The model under review builds one solid part; all positions refer to its coordinate system, in mm. A direction names the side the tool comes from. Round coordinates to 2 decimals unless told otherwise and drop trailing zeros. Order: outer loops, then holes, each group sorted by start corner. A loop starts at its lowest first (then second) coordinate and runs counter-clockwise, first axis right, second up. Notation, with made-up numbers: M 79,29.5 L 96,29.5 A26 cw 96,54.5 Z; hole C 25.25,73.5 d3. An arc over 180 degrees is marked long. Answer as CSV lines item,"result". Start each with the question number.
from build123d import *

# Parameters (mm, degrees)
SKETCH_1_W                  = 58
SKETCH_1_H                  = 103.5
EXTRUDE_1_DEPTH             = 12
HOLE_WIZARD_M4_1_D          = 3.3
SKETCH_5_R                  = 20
CUT_EXTRUDE_1_DEPTH         = 61.523239338
SKETCH_6_W                  = 58
SKETCH_6_H                  = 58
EXTRUDE_2_DEPTH             = 10
SKETCH_10_W                 = 48
SKETCH_10_H                 = 10
CUT_EXTRUDE_2_DEPTH         = 146
CHAMFER_1_SIZE              = 3
CUT_EXTRUDE_5_DEPTH         = 86.56320763
CUT_EXTRUDE_5_DEPTH_BACK    = 86.56320763
SKETCH_15_W                 = 130
SKETCH_15_H                 = 14
EXTRUDE_3_DEPTH             = 12
SKETCH_16_W                 = 40
SKETCH_16_H                 = 14
EXTRUDE_4_DEPTH             = 60
EXTRUDE_START               = -40
SKETCH_17_W                 = 12
SKETCH_17_H                 = 100
EXTRUDE_5_DEPTH             = 40
EXTRUDE_START_2             = -12
SKETCH_18_W                 = 72
SKETCH_18_H                 = 30
EXTRUDE_6_DEPTH             = 12
CHAMFER_2_SIZE              = 10
SKETCH_19_R                 = 22.248352005
SKETCH_19_R_2               = 12.5
EXTRUDE_7_DEPTH             = 8
CUT_EXTRUDE_6_DEPTH         = 158.012738337
CUT_EXTRUDE_6_DEPTH_BACK    = 158.012738337
HOLE_WIZARD_C_0_D           = 5.5
HOLE_WIZARD_C_0_CBORE_D     = 10
HOLE_WIZARD_C_0_CBORE_DEPTH = 5.5
CHAMFER_3_SIZE              = 10
HOLE_WIZARD_M4_2_D          = 3.3


with BuildPart() as part:
    # 草图1 → 凸台-拉伸1 (new body)
    with BuildSketch(Plane.XY):
        Rectangle(SKETCH_1_W, SKETCH_1_H)
    extrude(amount=EXTRUDE_1_DEPTH)

    # M4 螺纹孔1 (through all)
    with Locations(Plane(origin=(0, 0, 0), x_dir=(-1, 0, 0), z_dir=(0, 0, -1))):
        with Locations((-23.55, 46.8), (23.55, 46.8), (23.55, -0.3), (-23.55, -0.3)):
            Hole(HOLE_WIZARD_M4_1_D / 2)

    # 草图5 → 切除-拉伸1 (cut, through all)
    with BuildSketch(Plane(origin=(0, 0, 0), x_dir=(-1, 0, 0), z_dir=(0, 0, -1))):
        with Locations((0, 23.25)):
            Circle(SKETCH_5_R)
    extrude(amount=-CUT_EXTRUDE_1_DEPTH, mode=Mode.SUBTRACT)

    # 草图6 → 凸台-拉伸2 (add)
    with BuildSketch(Plane.XZ.offset(51.75)):
        with Locations((0, 29)):
            Rectangle(SKETCH_6_W, SKETCH_6_H)
    extrude(amount=EXTRUDE_2_DEPTH)

    # 草图10 → 切除-拉伸2 (cut)
    with BuildSketch(Plane(origin=(29, 0, 0), x_dir=(0, 0, -1), z_dir=(1, 0, 0))):
        with Locations((-36, -56.75)):
            Rectangle(SKETCH_10_W, SKETCH_10_H)
    extrude(amount=-CUT_EXTRUDE_2_DEPTH, mode=Mode.SUBTRACT)

    # 倒角1
    chamfer_1_edges = [part.edges().sort_by_distance(p)[0] for p in [
        (29, -61.75, 6),
        (-29, -61.75, 6),
        (-29, 51.75, 6),
        (29, 51.75, 6),
    ]]
    chamfer(chamfer_1_edges, length=CHAMFER_1_SIZE)

    # 草图14 → 切除-拉伸5 (cut, two sides: drawn at the far end of the back side and taken through both)
    with BuildSketch(Plane.ZY.offset(29).offset(-CUT_EXTRUDE_5_DEPTH_BACK)):
        Polygon((-205.249277876, -18.25), (-30, -18.25), (43.895682699, -18.25), (219.144960575, -18.25), (219.144960575, -368.748555752), (-205.249277876, -368.748555752), align=None)
    extrude(amount=CUT_EXTRUDE_5_DEPTH + CUT_EXTRUDE_5_DEPTH_BACK, mode=Mode.SUBTRACT)

    # 草图15 → 凸台-拉伸3 (add)
    with BuildSketch(Plane(origin=(0, 0, 0), x_dir=(-1, 0, 0), z_dir=(0, 0, -1))):
        with Locations((36, -25.25)):
            Rectangle(SKETCH_15_W, SKETCH_15_H)
    extrude(amount=-EXTRUDE_3_DEPTH)

    # 草图16 → 凸台-拉伸4 (add)
    with BuildSketch(Plane.XY.offset(12)):
        with Locations((-81, -25.25)):
            Rectangle(SKETCH_16_W, SKETCH_16_H)
    extrude(amount=EXTRUDE_4_DEPTH)

    # 草图17 → 凸台-拉伸5 (add)
    with BuildSketch(Plane.ZY.offset(101).offset(EXTRUDE_START)):
        with Locations((78, -68.25)):
            Rectangle(SKETCH_17_W, SKETCH_17_H)
    extrude(amount=EXTRUDE_5_DEPTH)

    # 草图18 → 凸台-拉伸6 (add)
    with BuildSketch(Plane(origin=(0, 0, 0), x_dir=(-1, 0, 0), z_dir=(0, 0, -1)).offset(EXTRUDE_START_2)):
        with Locations((65, -3.25)):
            Rectangle(SKETCH_18_W, SKETCH_18_H)
    extrude(amount=EXTRUDE_6_DEPTH)

    # 倒角2
    chamfer_2_edges = [part.edges().sort_by_distance(p)[0] for p in [
        (29, -32.25, 6),
    ]]
    chamfer(chamfer_2_edges, length=CHAMFER_2_SIZE)

    # 草图19 → 凸台-拉伸7 (add)
    with BuildSketch(Plane.XY.offset(12)):
        with Locations((0, 23.25)):
            Circle(SKETCH_19_R)
        with Locations((0, 23.25)):
            Circle(SKETCH_19_R_2, mode=Mode.SUBTRACT)
    extrude(amount=-EXTRUDE_7_DEPTH)

    # 草图20 → 切除-拉伸6 (cut, two sides: drawn at the far end of the back side and taken through both)
    with BuildSketch(Plane.XZ.offset(32.25).offset(-CUT_EXTRUDE_6_DEPTH_BACK)):
        Polygon((259.644501793, 12), (-52.844544679, 12), (-104.007164502, 12), (-416.496210973, 12), (-416.496210973, 636.978092943), (259.644501793, 636.978092943), align=None)
    extrude(amount=CUT_EXTRUDE_6_DEPTH + CUT_EXTRUDE_6_DEPTH_BACK, mode=Mode.SUBTRACT)

    # 打孔尺寸根据六角头螺栓 C 级的类型0 (through all)
    with Locations(Plane(origin=(0, 0, 0), x_dir=(-1, 0, 0), z_dir=(0, 0, -1))):
        with Locations((72.148493823, 215.242463417), (94, -26.25), (68, -26.25), (81, -10.25), (81, 1.75)):
            CounterBoreHole(HOLE_WIZARD_C_0_D / 2, HOLE_WIZARD_C_0_CBORE_D / 2, HOLE_WIZARD_C_0_CBORE_DEPTH)

    # 倒角3
    chamfer_3_edges = [part.edges().sort_by_distance(p)[0] for p in [
        (-101, 11.75, 6),
    ]]
    chamfer(chamfer_3_edges, length=CHAMFER_3_SIZE)

    # M4 螺纹孔2 (through all)
    with Locations(Plane.XY.offset(12)):
        with Locations((15, 8.25), (-15, 8.25), (-15, 38.25), (15, 38.25)):
            Hole(HOLE_WIZARD_M4_2_D / 2)


solid = part.part
Item 1: Consider section B-B (z = 2.75). State how many separate pieces and enclosed holes the cut face has, and give its area (3 significant figures).
Item 2: The part is to be moulded in two halves that separate along X. For faces 4 (the cylindrical face through (-98.619, -28.165, 2.712)), 5 (the flat face through (0, 51.75, 6)), 6 (the flat face through (-29, 31, 6)), say which applies: +X half, -X half, draft (parallel to the pull), parting line (faces both ways), or undercut.
Item 3: Consider section A-A (y = 23.25). State the section outline as (x, z) points.
Item 4: Wall thickness on probe 1 along Y at (x, z) = (-15, 6.5); probe 2 along Y at (x, z) = (-68, 7.75); probe 3 along Y at (x, z) = (-23.55, 4.75): over which ranges is each line inside the solid? List them lowest first. Write a range as [from, to].
Item 5: Consider section C-C (y = -26.25). State the section outline as (x, z) points, and give its area (3 significant figures).
Item 6: Consider section D-D (x = -68). State the section outline as (y, z) points, and give its area (3 significant figures).
Item 7: For pin 1 (1 mm diameter, centred on x = 9, y = 38, fed in from -Z); pin 2 (2 mm diameter, centred on x = 23.55, y = -0.3, fed in from -Z); pin 3 (1 mm diameter, centred on y = 13.5, z = 2, fed in from -X); pin 4 (9 mm diameter, centred on x = -68, y = -26.25, fed in from -Z), all flat-tipped, find the tip position at first contact; note any pin that passes through.
Item 8: Tool access review of faces 1 (the cylindrical face through (20, 23, 2)), 2 (the flat face through (29, 13, 6)), 3 (the flat face through (-60, 11.75, 6)): name each direction out of +Z, -Z, +X, -X, +Y, -Y from which nothing blocks a thin tool from reaching the whole face with its end or side.
Reported:
1,separate pieces,"1"
1,enclosed holes,"9"
1,area,"6,290 mm²"
2,face 4,"undercut"
2,face 5,"draft"
2,face 6,"-X half"
3,outline,"M -29,0 L -20,0 L -20,4 L -12.5,4 L -12.5,12 L -29,12 Z; M 12.5,4 L 20,4 L 20,0 L 29,0 L 29,12 L 12.5,12 Z"
4,probe 1,"y = [-32.25, 6.6], [9.9, 36.6], [39.9, 51.75]"
4,probe 2,"y = [-32.25, -29], [-23.5, 11.75]"
4,probe 3,"y = [-32.25, -1.95], [1.35, 45.15], [48.45, 51.75]"
5,outline,"M -101,0 L -99,0 L -99,5.5 L -96.75,5.5 L -96.75,12 L -101,12 Z; M -91.25,5.5 L -89,5.5 L -89,0 L -73,0 L -73,5.5 L -70.75,5.5 L -70.75,12 L -91.25,12 Z; M -65.25,5.5 L -63,5.5 L -63,0 L 25,0 L 25,12 L -65.25,12 Z"
5,area,"1,330 mm²"
6,outline,"M -32.25,0 L -31.25,0 L -31.25,5.5 L -29,5.5 L -29,12 L -32.25,12 Z; M -23.5,5.5 L -21.25,5.5 L -21.25,0 L 11.75,0 L 11.75,12 L -23.5,12 Z"
6,area,"437 mm²"
7,pin 1,"stops at z = 4"
7,pin 2,"passes through"
7,pin 3,"stops at x = -29"
7,pin 4,"stops at z = 5.5"
8,face 1,"-Z"
8,face 2,"+Z, -Z, +X, +Y, -Y"
8,face 3,"+Z, -Z, -X, +Y"
